from build123d import *

# Parameters (mm, degrees)
SKETCH1_R           = 3.1
BOSS_EXTRUDE2_DEPTH = 6


with BuildPart() as part:
    # Sketch1 → Boss-Extrude2 (new body)
    with BuildSketch(Plane(origin=(0, 0, 0), x_dir=(1, 0, 0), z_dir=(0, 1, 0))):
        with BuildLine():
            Line((-7.442631645, 168.908075373), (-7.442631645, 256.750012922))
            ThreePointArc((-7.442631645, 256.750012922), (12.557368355, 276.750012922), (32.557368355, 256.750012922))
            Line((32.557368355, 256.750012922), (32.557368355, 168.908075373))
            ThreePointArc((32.557368355, 168.908075373), (67.390763371, 38.908075373), (162.557368355, -56.258529611))
            Line((162.557368355, -56.258529611), (238.63071779, -100.179498385))
            ThreePointArc((238.63071779, -100.179498385), (245.951225865, -127.500006461), (218.63071779, -134.820514537))
            Line((218.63071779, -134.820514537), (142.557368355, -90.899545762))
            ThreePointArc((142.557368355, -90.899545762), (12.557368355, -56.066150746), (-117.442631645, -90.899545762))
            Line((-117.442631645, -90.899545762), (-193.51598108, -134.820514537))
            ThreePointArc((-193.51598108, -134.820514537), (-220.836485566, -127.499986835), (-213.515954749, -100.179483183))
            Line((-213.515954749, -100.179483183), (-137.442631645, -56.258529611))
            ThreePointArc((-137.442631645, -56.258529611), (-42.276026661, 38.908075373), (-7.442631645, 168.908075373))
        make_face()
        with Locations(Location((12.557368355, 7.25, 0), (0, 0, 270))):
            Circle(SKETCH1_R, mode=Mode.SUBTRACT)
        with BuildLine():
            Line((5.830127019, -0.098076211), (-202.015969889, -120.098076211))
            ThreePointArc((-202.015969889, -120.098076211), (-206.114046101, -119), (-205.015969889, -114.901923789))
            Line((-205.015969889, -114.901923789), (2.830127019, 5.098076211))
            ThreePointArc((2.830127019, 5.098076211), (6.92820323, 4), (5.830127019, -0.098076211))
        make_face(mode=Mode.SUBTRACT)
        with BuildLine():
            Line((22.284609691, 5.098076211), (230.130706599, -114.901923789))
            ThreePointArc((230.130706599, -114.901923789), (231.22878281, -119), (227.130706599, -120.098076211))
            Line((227.130706599, -120.098076211), (19.284609691, -0.098076211))
            ThreePointArc((19.284609691, -0.098076211), (18.186533479, 4), (22.284609691, 5.098076211))
        make_face(mode=Mode.SUBTRACT)
        with BuildLine():
            Line((9.557368355, 16.75), (9.557368355, 256.75))
            ThreePointArc((9.557368355, 256.75), (12.557368355, 259.75), (15.557368355, 256.75))
            Line((15.557368355, 256.75), (15.557368355, 16.75))
            ThreePointArc((15.557368355, 16.75), (12.557368355, 13.75), (9.557368355, 16.75))
        make_face(mode=Mode.SUBTRACT)
    extrude(amount=BOSS_EXTRUDE2_DEPTH)


solid = part.part
Design review of the part built by this model. Coordinates are the model's own, in mm. A direction names the side the tool comes from. Give positions to 0.01 mm unless a question says otherwise; leave off trailing zeros. Order: outer loops, then holes, each group sorted by start corner. A loop starts at its lowest first (then second) coordinate and runs counter-clockwise, first axis right, second up. Notation, with made-up numbers: (53.5, -8) - (67.5, -8) arc R29 cw to (67.5, 23) - close; hole circle Ø1 at (3, 80). An arc over 180 degrees is marked (long way). Write item = value, one per line. Start each with the question number.
Q1. We need section B-B on x = 213. State the section outline as (y, z) points, plus the area to 3 significant figures.
Q2. We need section C-C on z = 23. State the section outline as (x, y) points.
Q3. Tool access review of faces 1 (the face through (-102.548, 2.958, 55.742)), 2 (the face through (181.13, 2.96, 113.17)), 3 (the face through (14, 0, 6)): name each direction out of +Z, -Z, +X, -X, +Y, -Y from which nothing blocks a thin tool from reaching the whole face with its end or side.
Q4. To check wall thickness, follow L1, parallel to X at y = 2.85, z = -212; L2, parallel to X at y = 0.35, z = 104; L3, parallel to Z at x = 91.5, y = 3.45. State the ranges of each line that lie inside material, in increasing order. Write a range as from..to.
Q5. We need section D-D on y = 1.35. State the section outline as (x, z) points, plus the area to 3 significant figures.
Q6. Mouldability with a two-part tool opening along Z and no side actions: class faces 4 (the face through (124.663, 2.958, 60.938)), 5 (the face through (12.118, 2.958, -276.745)), 6 (the face through (124.75, 2.96, 54.06)), 7 (the face through (14, 6, 6)) as released by +Z, released by -Z, zero draft, split by the parting line, or undercut.
Q7. We need section A-A on z = -226. State the section outline as (x, y) points.
Q8. Clearance check with flat-ended pins moving along their axes: pin 1 Ø7 at (x, z) = (12.56, -7.25) entering from -Y; pin 2 Ø1.5 at (x, y) = (142.5, 1) entering from -Z; pin 3 Ø3 at (y, z) = (4.5, -234) entering from +X. State where each tip first meets the part, or that it passes through.
Working result:
q1.outline = (0, 85.38) - (6, 85.38) - (6, 105.01) - (0, 105.01) - close; (0, 111.94) - (6, 111.94) - (6, 131.57) - (0, 131.57) - close
q1.area = 236 mm²
q2.outline = (-92.03, 0) - (-45.84, 0) - (-45.84, 6) - (-92.03, 6) - close; (-33.84, 0) - (58.95, 0) - (58.95, 6) - (-33.84, 6) - close; (70.95, 0) - (117.14, 0) - (117.14, 6) - (70.95, 6) - close
q3.face_1 = +Y, -Y
q3.face_2 = +Z, +Y, -Y
q3.face_3 = +Z, -Z, +X, -X, -Y
q4.L1 = -7.44..9.56, 15.56..32.56
q4.L2 = -218.27..-186.13, -174.13..-140.13, 165.25..199.25, 211.25..243.39
q4.L3 = -4.06..34.86, 41.79..68.34
q5.outline = (-213.52, 100.18) - (-137.44, 56.26) arc R260 cw to (-7.44, -168.91) - (-7.44, -256.75) arc R20 ccw to (32.56, -256.75) - (32.56, -168.91) arc R260 cw to (162.56, 56.26) - (238.63, 100.18) arc R20 ccw to (218.63, 134.82) - (142.56, 90.9) arc R260 cw to (-117.44, 90.9) - (-193.52, 134.82) arc R20 ccw to start; hole (-205.02, 114.9) - (2.83, -5.1) arc R3 ccw to (5.83, 0.1) - (-202.02, 120.1) arc R3 ccw to start; hole circle Ø6.2 at (12.56, -7.25); hole (9.56, -256.75) arc R3 ccw to (15.56, -256.75) - (15.56, -16.75) arc R3 ccw to (9.56, -16.75) - close; hole (19.28, 0.1) arc R3 ccw to (22.28, -5.1) - (230.13, 114.9) arc R3 ccw to (227.13, 120.1) - close
q5.area = 37,600 mm²
q6.face_4 = undercut
q6.face_5 = released by -Z
q6.face_6 = undercut
q6.face_7 = zero draft
q7.outline = (-7.44, 0) - (9.56, 0) - (9.56, 6) - (-7.44, 6) - close; (15.56, 0) - (32.56, 0) - (32.56, 6) - (15.56, 6) - close
q8.pin_1 = 0
q8.pin_2 = 42.89
q8.pin_3 = 32.56
